```python
from build123d import *

# Parameters (mm, degrees)
BOSS_EXTRUDE1_DEPTH   = 110
CHAMFER1_SIZE         = 2
CUT_EXTRUDE1_DEPTH    = 150.127637408
M6_TAPPED_HOLE1_D     = 5
M6_TAPPED_HOLE1_DEPTH = 10.497848452
M6_TAPPED_HOLE1_TIP   = 1.502151548


with BuildPart() as part:
    # Sketch1 → Boss-Extrude1 (new body)
    with BuildSketch(Plane.XY):
        Polygon((-38.601194786, 51.777777778), (-38.601194786, -53.222222222), (-2.601194786, -53.222222222), (-2.601194786, -41.222222222), (-26.601194786, -41.222222222), (-26.601194786, 51.777777778), align=None)
    extrude(amount=BOSS_EXTRUDE1_DEPTH)

    # Chamfer1
    chamfer1_edges = [part.edges().sort_by_distance(p)[0] for p in [
        (-38.601194786, -53.222222222, 55),
        (-2.601194786, -47.222222222, 110),
        (-32.601194786, 51.777777778, 110),
        (-2.601194786, -47.222222222, 0),
        (-32.601194786, 51.777777778, 0),
    ]]
    chamfer(chamfer1_edges, length=CHAMFER1_SIZE)

    # Sketch2 → Cut-Extrude1 (cut, through all)
    with BuildSketch(Plane(origin=(0, -41.222222222, 0), x_dir=(1, 0, 0), z_dir=(0, 1, 0))):
        with BuildLine():
            Line((-15.601194786, -97.5), (-15.601194786, -82.5))
            ThreePointArc((-15.601194786, -82.5), (-12.601194786, -79.5), (-9.601194786, -82.5))
            Line((-9.601194786, -82.5), (-9.601194786, -97.5))
            ThreePointArc((-9.601194786, -97.5), (-12.601194786, -100.5), (-15.601194786, -97.5))
        make_face()
        with BuildLine():
            Line((-15.601194786, -12.5), (-15.601194786, -27.5))
            ThreePointArc((-15.601194786, -27.5), (-12.601194786, -30.5), (-9.601194786, -27.5))
            Line((-9.601194786, -27.5), (-9.601194786, -12.5))
            ThreePointArc((-9.601194786, -12.5), (-12.601194786, -9.5), (-15.601194786, -12.5))
        make_face()
    extrude(amount=-CUT_EXTRUDE1_DEPTH, mode=Mode.SUBTRACT)

    # M6 Tapped Hole1
    with Locations(Plane(origin=(0, 51.777777778, 0), x_dir=(1, 0, 0), z_dir=(0, 1, 0))):
        with Locations((-32.601194786, -99), (-32.601194786, -11)):
            Hole(M6_TAPPED_HOLE1_D / 2, depth=M6_TAPPED_HOLE1_DEPTH)
            with Locations((0, 0, -(M6_TAPPED_HOLE1_DEPTH + M6_TAPPED_HOLE1_TIP / 2))):  # 118° drill point
                Cone(0, M6_TAPPED_HOLE1_D / 2, M6_TAPPED_HOLE1_TIP, mode=Mode.SUBTRACT)


solid = part.part
```
For this review, take the finished solid that the model builds, in its own axes (mm). A direction names the side the tool comes from. Give positions to 0.01 mm unless a question says otherwise; leave off trailing zeros. Loops run counter-clockwise (first coordinate to the right, second up) from the corner with the lowest first, then second, coordinate; pieces in that order, holes last. Notation, with made-up numbers: M 74,28.5 L 83,28.5 A34 cw 83,59.5 Z; hole C -1,-4 d8. An arc over 180 degrees is marked long. One line per item, written item: value. Start each with the question number.
Q1. Add section B-B (x = -11). Give the boundary of the cut face in (y, z), and give its area (3 significant figures).
Q2. Add section D-D (x = -18.5). Give the boundary of the cut face in (y, z), and give its area (3 significant figures).
Q3. Machinability: for faces 4 (the face through (-29, -12, 0)), 5 (the face through (-15.601, -47, 20)), 6 (the face through (-38.601, 1, 54)), 7 (the face through (-34.986, 46.455, 98.249)), 8 (the face through (-26.601, 5, 54)), which of the approach directions +Z, -Z, +X, -X, +Y, -Y give a long, thin tool a straight path to every point of the face, cutting with its end or side? Answer none if there is none.
Q4. Add section C-C (y = -4.5). Give the boundary of the cut face in (x, z), and give its area (3 significant figures).
Q5. Clearance check with flat-ended pins moving along their axes: pin 1 Ø1.5 at (y, z) = (-12.5, 20.5) entering from +X; pin 2 Ø12 at (x, z) = (-17, 41) entering from +Y; pin 3 Ø4.5 at (x, z) = (-32.6, 11) entering from +Y. State where each tip first meets the part, or that it passes through.
Q6. Draft analysis for pull direction X (two halves, no side actions). For faces 1 (the face through (-2.601, -47, 54)), 2 (the face through (-29, -12, 110)), 3 (the face through (-9.601, -47, 90)), state which applies: released by +X, released by -X, zero draft, split by the parting line, or undercut.
Q7. Add section A-A (z = 68.5). Give the boundary of the cut face in (x, y), and give its area (3 significant figures).
Q8. For L1, parallel to X at y = 49.75, z = 11; L2, parallel to Z at x = -10, y = -42; L3, parallel to X at y = 0.5, z = 61, list the stretches that pass through material, from the lowest coordinate up.
Reply:
1. outline: M -53.22,0 L -41.22,0 L -41.22,9.96 L -53.22,9.96 Z; M -53.22,30.04 L -41.22,30.04 L -41.22,79.96 L -53.22,79.96 Z; M -53.22,100.04 L -41.22,100.04 L -41.22,110 L -53.22,110 Z
1. area: 838 mm²
2. outline: M -53.22,0 L -41.22,0 L -41.22,110 L -53.22,110 Z
2. area: 1,320 mm²
3. face 4: -Z, +X, -X, +Y, -Y
3. face 5: +Y, -Y
3. face 6: +Z, -Z, -X, +Y, -Y
3. face 7: +Y
3. face 8: +Z, -Z, +X, +Y
4. outline: M -38.6,0 L -26.6,0 L -26.6,110 L -38.6,110 Z
4. area: 1,320 mm²
5. pin 1: x = -26.6
5. pin 2: y = -41.22
5. pin 3: y = 41.13
6. face 1: released by +X
6. face 2: zero draft
6. face 3: undercut
7. outline: M -38.6,-51.22 L -36.6,-53.22 L -2.6,-53.22 L -2.6,-41.22 L -26.6,-41.22 L -26.6,51.78 L -38.6,51.78 Z
7. area: 1,550 mm²
8. L1: -38.6 to -35.1, -30.1 to -26.6
8. L2: 0 to 11.01, 28.99 to 81.01, 98.99 to 110
8. L3: -38.6 to -26.6
